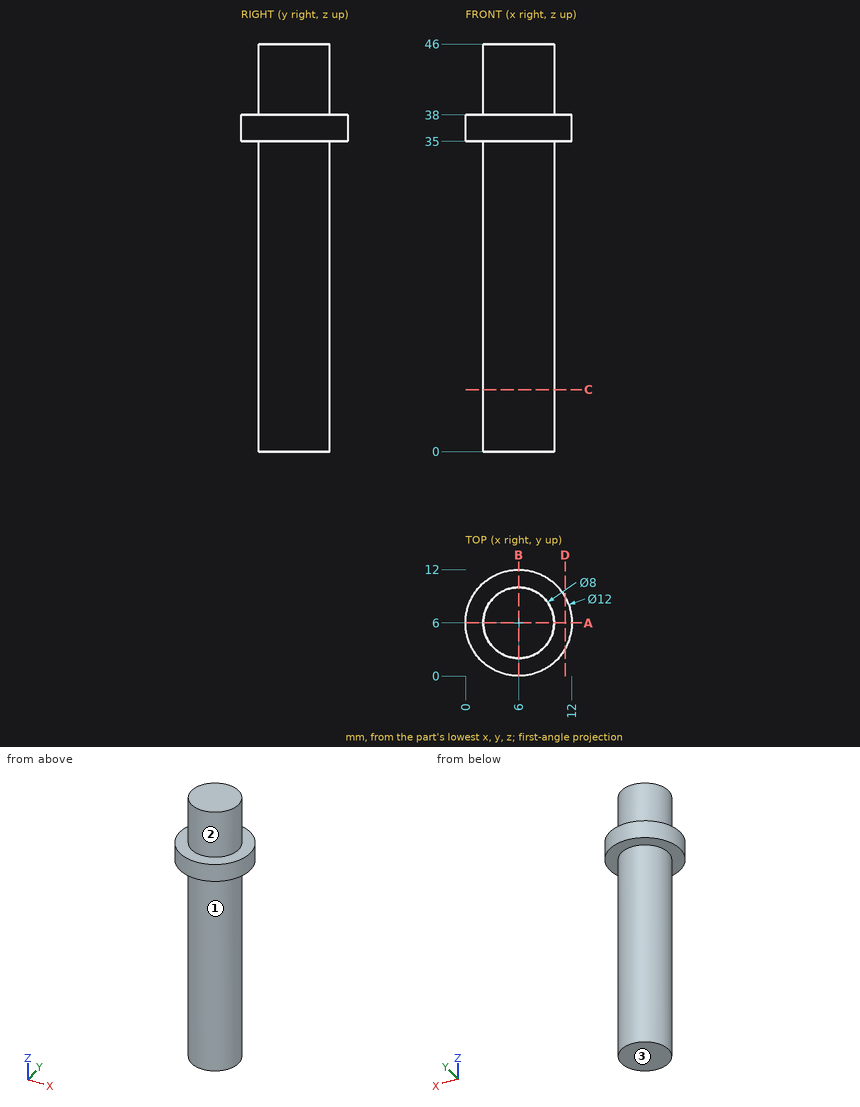
Print and shaded views of the part. All mm, measured from the part's lowest x, y and z. A direction names the side the tool comes from. Coordinates: 2 decimals unless noted, no trailing zeros. Loops run counter-clockwise (first coordinate to the right, second up) from the corner with the lowest first, then second, coordinate; pieces in that order, holes last. Notation, with made-up numbers: (5.25, 2.25) -> (15.25, 2.25) arc R14 cw to (15.25, 10.25) -> close; hole circle Ø2 at (86.5, 62). An arc over 180 degrees is marked (long way). Use a Markdown table: item, result. Add a question column.
Item 1: Which spindle directions (+Z, -Z, +X, -X, +Y, -Y) get a long thin tool onto all of the face, cutting with end or side? Do the marked faces 1, 2 and 3. Say none if no direction does.
Item 2: Band-saw the part on C-C on z = 7. Write the cut outline in (x, y), plus the area to 3 significant figures.
Item 3: Flat gauge pins, fed straight in: P1, Ø4, axis at y = 3.5, z = 32, coming from the -X side; P2, Ø2, axis at y = 8, z = 5.5, coming from the +X side; P3, Ø6, axis at x = 6, z = 9, coming from the -Y side. Where does each tip first touch, or does it go through?
Item 4: Probe probe 1 along Z at (x, y) = (1.5, 3.75); probe 2 along X at (y, z) = (4, 34.5); probe 3 along Y at (x, z) = (3.25, 16.5). List the from-to ranges inside material, lowest first.
Item 5: Band-saw the part on A-A on y = 6. Write the cut outline in (x, z).
Item 6: Band-saw the part on D-D on x = 11.25. Write the cut outline in (y, z).
Geometry says:
| question | item | result |
|---|---|---|
| 1 | face 1 | -Z |
| 1 | face 2 | +Z |
| 1 | face 3 | -Z, +X, -X, +Y, -Y |
| 2 | outline | circle Ø8 at (6, 6) |
| 2 | area | 50.3 mm² |
| 3 | P1 | x = 2.03 |
| 3 | P2 | x = 9.87 |
| 3 | P3 | y = 2 |
| 4 | probe 1 | 35 to 38 |
| 4 | probe 2 | 2.54 to 9.46 |
| 4 | probe 3 | 3.1 to 8.9 |
| 5 | outline | (0, 35) -> (2, 35) -> (2, 0) -> (10, 0) -> (10, 35) -> (12, 35) -> (12, 38) -> (10, 38) -> (10, 46) -> (2, 46) -> (2, 38) -> (0, 38) -> close |
| 6 | outline | (3.1, 35) -> (8.9, 35) -> (8.9, 38) -> (3.1, 38) -> close |
